Here's how the part is built. I have some questions about the finished solid (model axes, mm). Face numbers are marked on the shaded views. A direction names the side the tool comes from. Round coordinates to 2 decimals unless told otherwise and drop trailing zeros. Write each loop counter-clockwise with the first axis right and the second up, starting at its lowest first coordinate (ties: lowest second). Pieces come first, ordered by that corner, then holes. Notation, with made-up numbers: (10.25, 11) -> (40.25, 11) arc R13 ccw to (40.25, 16) -> close; hole circle Ø6 at (61.5, -2). An arc over 180 degrees is marked (long way). Put each result on its own line as item: value. Start each with the question number.
1. Suppose I cut it at C-C (x = 1.2). Please give me the cut outline in (y, z).
2. Suppose I cut it at B-B (z = 1.15). Please give me the cut outline in (x, y), then the cut area to 3 significant figures.
3. Suppose I cut it at D-D (x = 0). Please give me the cut outline in (y, z).
4. Suppose I cut it at A-A (y = -13). Please give me the cut outline in (x, z).
5. We'd pull the mould along X, two halves only. Please class the marked faces 4, 5 and 6: +X half, -X half, draft (parallel to the pull), parting line (faces both ways), or undercut.
6. Which directions (+Z, -Z, +X, -X, +Y, -Y) give clear straight access to the entire face, cutting with the end or side of a thin tool? Please do the marked faces 1, 2 and 3.
7. I need wall thicknesses on probe 1 along X at (y, z) = (13.75, 0.7); probe 2 along Y at (x, z) = (0.1, 0.35); probe 3 along X at (y, z) = (-11.5, 0.5). Which ranges of each line are inside material? Lowest first, please. Write a range as from..to.
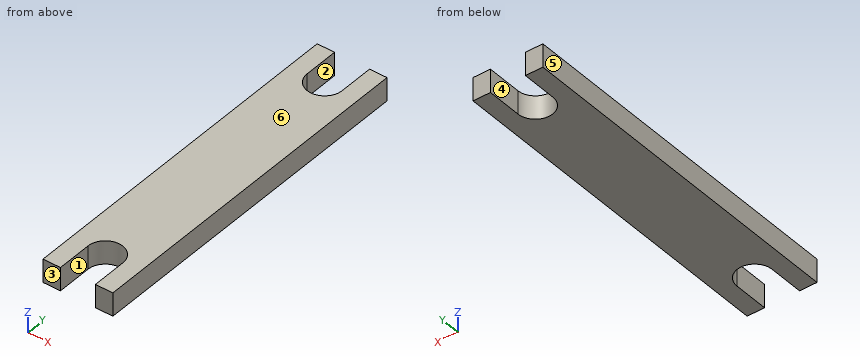
```python
from build123d import *

# Parameters (mm, degrees)
BOSS_EXTRUDE1_DEPTH = 2


with BuildPart() as part:
    # Sketch1 → Boss-Extrude1 (new body)
    with BuildSketch(Plane.XY):
        with BuildLine():
            Line((3, 15), (3, -15))
            Line((3, -15), (1.5, -15))
            Line((1.5, -15), (1.5, -12))
            ThreePointArc((1.5, -12), (0, -10.5), (-1.5, -12))
            Line((-1.5, -12), (-1.5, -15))
            Line((-1.5, -15), (-3, -15))
            Line((-3, -15), (-3, 15))
            Line((-3, 15), (-1.5, 15))
            Line((-1.5, 15), (-1.5, 12))
            ThreePointArc((-1.5, 12), (0, 10.5), (1.5, 12))
            Line((1.5, 12), (1.5, 15))
            Line((1.5, 15), (3, 15))
        make_face()
    extrude(amount=BOSS_EXTRUDE1_DEPTH)


solid = part.part
```
Verdict:
1. outline: (-11.1, 0) -> (11.1, 0) -> (11.1, 2) -> (-11.1, 2) -> close
2. outline: (-3, -15) -> (-1.5, -15) -> (-1.5, -12) arc R1.5 cw to (1.5, -12) -> (1.5, -15) -> (3, -15) -> (3, 15) -> (1.5, 15) -> (1.5, 12) arc R1.5 cw to (-1.5, 12) -> (-1.5, 15) -> (-3, 15) -> close
2. area: 155 mm^2
3. outline: (-10.5, 0) -> (10.5, 0) -> (10.5, 2) -> (-10.5, 2) -> close
4. outline: (-3, 0) -> (-1.5, 0) -> (-1.5, 2) -> (-3, 2) -> close; (1.5, 0) -> (3, 0) -> (3, 2) -> (1.5, 2) -> close
5. face 4: undercut
5. face 5: -X half
5. face 6: draft
6. face 1: +Z, -Z, -Y
6. face 2: +Z, -Z, +Y
6. face 3: +Z, -Z, +X, -X, -Y
7. probe 1: x = -3..-1.5, 1.5..3
7. probe 2: y = -10.5..10.5
7. probe 3: x = -3..-1.41, 1.41..3
